Design review of the part built by this model. Coordinates are the model's own, in mm. Face numbers are marked on the shaded views. A direction names the side the tool comes from. Give positions to 0.01 mm unless a question says otherwise; leave off trailing zeros. Write each loop counter-clockwise with the first axis right and the second up, starting at its lowest first coordinate (ties: lowest second). Pieces come first, ordered by that corner, then holes. Notation, with made-up numbers: (81.25, -35.75) -> (105.25, -35.75) arc R22 cw to (105.25, -25.75) -> close; hole circle Ø6 at (61, 48). An arc over 180 degrees is marked (long way). Use CSV: the item, a comma, the result in double quotes.
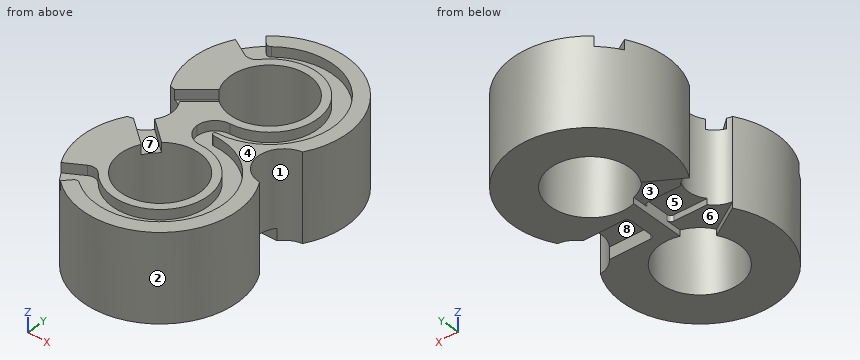
```python
from build123d import *

# Parameters (mm, degrees)
SKETCH_1_R             = 10
EXTRUDE_1_DEPTH        = 22
CUT_EXTRUDE_1_DEPTH    = 2.5
FILLET_1_R             = 1
FILLET_2_R             = 2.5
FILLET_1_OF_MIRROR_1_R = 1
FILLET_2_OF_MIRROR_1_R = 2.5
CUT_EXTRUDE_2_DEPTH    = 2.5
CUT_EXTRUDE_3_DEPTH    = 1.5
SKETCH_5_W             = 15.539550215
SKETCH_5_H             = 8
CUT_EXTRUDE_4_DEPTH    = 1.5
SKETCH_6_W             = 13.998675607
SKETCH_6_H             = 8
CUT_EXTRUDE_5_DEPTH    = 3
FILLET_3_R             = 1


with BuildPart() as part:
    # 草图1 → 凸台-拉伸1 (new body)
    with BuildSketch(Plane.XY):
        with BuildLine():
            ThreePointArc((16.714762364, 6.456757539), (0, 36), (-16.714762364, 6.456757539))
            ThreePointArc((-16.714762364, 6.456757539), (-10.963282289, 0), (-16.714762364, -6.456757539))
            ThreePointArc((-16.714762364, -6.456757539), (0, -36), (16.714762364, -6.456757539))
            ThreePointArc((16.714762364, -6.456757539), (10.963282289, 0), (16.714762364, 6.456757539))
        make_face()
        with Locations((0, 16.5)):
            Circle(SKETCH_1_R, mode=Mode.SUBTRACT)
        with Locations((0, -16.5)):
            Circle(SKETCH_1_R, mode=Mode.SUBTRACT)
    extrude(amount=EXTRUDE_1_DEPTH)

    # 草图2 → 切除-拉伸1 (cut)
    with BuildSketch(Plane.XY.offset(22)):
        with BuildLine():
            Line((-10.392304845, 22.5), (-20.279992845, 28.208659328))
            Line((-20.279992845, 28.208659328), (-16.120486586, 34.166566083))
            Line((-16.120486586, 34.166566083), (-10.784713231, 28.319050745))
            ThreePointArc((-10.784713231, 28.319050745), (14.918190439, 22.283389494), (0, 0.5))
            ThreePointArc((0, 0.5), (-0.353553391, 0.353553391), (-0.5, 0))
            Line((-0.5, 0), (-4.5, 0))
            ThreePointArc((-4.5, 0), (-3.181980515, 3.181980515), (0, 4.5))
            ThreePointArc((0, 4.5), (10.392304845, 22.5), (-10.392304845, 22.5))
        make_face()
    cut_extrude_1 = extrude(amount=-CUT_EXTRUDE_1_DEPTH, mode=Mode.SUBTRACT)

    # 圆角1
    fillet_1_edges = [part.edges().sort_by_distance(p)[0] for p in [
        (-10.784713231, 28.319050745, 20.75),
    ]]
    fillet(fillet_1_edges, radius=FILLET_1_R)

    # 圆角2
    fillet_2_edges = [part.edges().sort_by_distance(p)[0] for p in [
        (-10.392304845, 22.5, 20.75),
    ]]
    fillet(fillet_2_edges, radius=FILLET_2_R)

    # 镜向1: 切除-拉伸1 across plane
    add(cut_extrude_1.mirror(Plane.ZX), mode=Mode.SUBTRACT)

    # 圆角1 of 镜向1
    fillet_1_of_mirror_1_edges = [part.edges().sort_by_distance(p)[0] for p in [
        (-10.784713231, -28.319050745, 20.75),
    ]]
    fillet(fillet_1_of_mirror_1_edges, radius=FILLET_1_OF_MIRROR_1_R)

    # 圆角2 of 镜向1
    fillet_2_of_mirror_1_edges = [part.edges().sort_by_distance(p)[0] for p in [
        (-10.392304845, -22.5, 20.75),
    ]]
    fillet(fillet_2_of_mirror_1_edges, radius=FILLET_2_OF_MIRROR_1_R)

    # 草图3 → 切除-拉伸2 (cut)
    with BuildSketch(Plane.XY.offset(22)):
        Polygon((-7.454777322, 12.855513677), (-16.290741775, 5.441259163), (-13.719591337, 2.377081391), (-4.883626883, 9.791335905), align=None)
        Polygon((-13.453227562, -2.600587136), (-5.167237951, -9.553357963), (-7.738388389, -12.617535735), (-16.448259291, -5.309086274), align=None)
    extrude(amount=-CUT_EXTRUDE_2_DEPTH, mode=Mode.SUBTRACT)

    # 草图4 → 切除-拉伸3 (cut)
    with BuildSketch(Plane(origin=(0, 0, 0), x_dir=(-1, 0, 0), z_dir=(0, 0, -1))):
        Polygon((3, 14.697418143), (16.714762364, 6.456757539), (16.714762364, -6.456757539), (3, -14.697418143), align=None)
    extrude(amount=-CUT_EXTRUDE_3_DEPTH, mode=Mode.SUBTRACT)

    # 草图5 → 切除-拉伸4 (cut)
    with BuildSketch(Plane(origin=(0, 0, 1.5), x_dir=(-1, 0, 0), z_dir=(0, 0, -1))):
        with Locations((10.769775108, 0)):
            Rectangle(SKETCH_5_W, SKETCH_5_H)
    extrude(amount=-CUT_EXTRUDE_4_DEPTH, mode=Mode.SUBTRACT)

    # 草图6 → 切除-拉伸5 (cut)
    with BuildSketch(Plane(origin=(0, 0, 0), x_dir=(-1, 0, 0), z_dir=(0, 0, -1))):
        with Locations((-7.999337804, 0)):
            Rectangle(SKETCH_6_W, SKETCH_6_H)
    extrude(amount=-CUT_EXTRUDE_5_DEPTH, mode=Mode.SUBTRACT)

    # 圆角3
    fillet_3_edges = [part.edges().sort_by_distance(p)[0] for p in [
        (-3, 4, 2.25),
        (-3, -4, 2.25),
        (1, 4, 1.5),
        (1, -4, 1.5),
    ]]
    fillet(fillet_3_edges, radius=FILLET_3_R)


solid = part.part
```
(1) Mouldability with a two-part tool opening along X and no side actions: class the marked faces 1, 2, 3 and 4 as +X half, -X half, draft (parallel to the pull), parting line (faces both ways), or undercut.
Established:
face 1,"+X half"
face 2,"parting line"
face 3,"undercut"
face 4,"draft"
(2) Take a section at A-A (y = 16.5). Write out the cut boundary in (x, z), then the cut area to 3 significant figures.
Established:
outline,"(-19.5, 0) -> (-10, 0) -> (-10, 22) -> (-19.5, 22) -> close; (10, 0) -> (19.5, 0) -> (19.5, 22) -> (16, 22) -> (16, 19.5) -> (12, 19.5) -> (12, 22) -> (10, 22) -> close"
area,"408 mm2"
(3) Take a section at B-B (x = 6). State how many separate pieces and enclosed holes the cut face has, then the cut area to 3 significant figures.
Established:
separate pieces,"3"
enclosed holes,"0"
area,"770 mm2"
(4) For line 1 along Y through (x, z) = (0, 9.25); line 2 along X through (y, z) = (16.5, 20.15); line 3 along X through (y, z) = (-16.5, 11.75), list the stretches that pass through material, from the lowest coordinate up. Write a range as [from, to].
Established:
line 1,"y = [-36, -26.5], [-6.5, 6.5], [26.5, 36]"
line 2,"x = [-19.5, -10], [10, 12], [16, 19.5]"
line 3,"x = [-19.5, -10], [10, 19.5]"
(5) Tool access review of the marked faces 5, 6, 7 and 8: name each direction out of +Z, -Z, +X, -X, +Y, -Y from which nothing blocks a thin tool from reaching the whole face with its end or side.
Established:
face 5,"-Z, -X"
face 6,"-Z"
face 7,"+Z"
face 8,"-Z, +X"
(6) Take a section at C-C (z = 15.25). Write out the cut boundary in (x, y), then the cut area to 3 significant figures.
Established:
outline,"(-16.71, -6.46) arc R19.5 ccw (long way) to (16.71, -6.46) arc R6.5 cw to (16.71, 6.46) arc R19.5 ccw (long way) to (-16.71, 6.46) arc R6.5 cw to start; hole circle Ø20 at (0, -16.5); hole circle Ø20 at (0, 16.5)"
area,"1,630 mm2"
(7) Clearance check with flat-ended pins moving along their axes: pin 1 (5 mm diameter, centred on y = -18, z = 16, fed in from -X); pin 2 (1.5 mm diameter, centred on y = -20, z = 2.5, fed in from -X); pin 3 (4 mm diameter, centred on x = 14, z = 14.5, fed in from +Y); pin 4 (1.6 mm diameter, centred on x = -8.5, z = 2, fed in from +Y). State where each tip first meets the part, or that it passes through.
Established:
pin 1,"stops at x = -19.5"
pin 2,"stops at x = -19.31"
pin 3,"stops at y = 31.87"
pin 4,"stops at y = 34.42"
(8) Take a section at D-D (x = 17.5). Write out the cut boundary in (y, z), then the cut area to 3 significant figures.
Established:
outline,"(-25.1, 0) -> (-7.9, 0) -> (-7.9, 22) -> (-25.1, 22) -> close; (7.9, 0) -> (25.1, 0) -> (25.1, 22) -> (7.9, 22) -> close"
area,"757 mm2"
